from build123d import *

# Parameters (mm, degrees)
SKETCH1_R           = 17.5
BOSS_EXTRUDE1_DEPTH = 200
SKETCH3_OUTSIDE_W   = 78.206
SKETCH3_OUTSIDE_H   = 78.206
SKETCH3_OUTSIDE_R   = 12
CUT_EXTRUDE1_DEPTH  = 24
SKETCH4_W           = 220
SKETCH4_H           = 26
BOSS_EXTRUDE2_DEPTH = 23
CHAMFER1_SIZE       = 10


with BuildPart() as part:
    # Sketch1 → Boss-Extrude1 (new body)
    with BuildSketch(Plane.XY):
        Circle(SKETCH1_R)
    extrude(amount=BOSS_EXTRUDE1_DEPTH)

    # Sketch3 outside → Cut-Extrude1 (cut)
    with BuildSketch(Plane.XY.offset(200)):
        Rectangle(SKETCH3_OUTSIDE_W, SKETCH3_OUTSIDE_H)
        Circle(SKETCH3_OUTSIDE_R, mode=Mode.SUBTRACT)
    extrude(amount=-CUT_EXTRUDE1_DEPTH, mode=Mode.SUBTRACT)

    # Sketch4 → Boss-Extrude2 (add)
    with BuildSketch(Plane.XY.offset(200)):
        Rectangle(SKETCH4_W, SKETCH4_H)
    extrude(amount=BOSS_EXTRUDE2_DEPTH)

    # Chamfer1
    chamfer1_edges = [part.edges().sort_by_distance(p)[0] for p in [
        (-110, 0, 223),
        (110, 0, 223),
    ]]
    chamfer(chamfer1_edges, length=CHAMFER1_SIZE)


solid = part.part
The model under review builds one solid part; all positions refer to its coordinate system, in mm. A direction names the side the tool comes from. Give positions to 0.01 mm unless a question says otherwise; leave off trailing zeros. Loops run counter-clockwise (first coordinate to the right, second up) from the corner with the lowest first, then second, coordinate; pieces in that order, holes last. Notation, with made-up numbers: (67, 3.5) -> (125, 3.5) arc R12 cw to (125, 23.5) -> close; hole circle Ø7 at (75.5, -26.5). An arc over 180 degrees is marked (long way). Put each result on its own line as item: value. Start each with the question number.
1. We need section B-B on y = 5. State the section outline as (x, z) points.
2. Mouldability with a two-part tool opening along Z and no side actions: class faces 1 (the face through (-11.99, 0.53, 188.17)), 2 (the face through (0, 0, 0)), 3 (the face through (-13.887, -10.648, 86.768)) as released by +Z, released by -Z, zero draft, split by the parting line, or undercut.
3. For faces 4 (the face through (-105, 0, 218)), 5 (the face through (-12, -4, 176)), list the 3-axis set-ups (+Z, -Z, +X, -X, +Y, -Y) from which the entire face can be reached by the end or side of a thin tool; tool diameter is ignored.
4. We need section A-A on x = 0. State the section outline as (y, z) points.
5. We need section C-C on z = 125. State the section outline as (x, y) points.
6. Clearance check with flat-ended pins moving along their axes: P1, Ø1, axis at x = 78, y = -4, coming from the -Z side; P2, Ø11.5, axis at x = 14.5, z = 215.5, coming from the -Y side; P3, Ø1, axis at y = -13.5, z = 174, coming from the +X side. State where each tip first meets the part, or that it passes through.
7. We need section D-D on x = 34. State the section outline as (y, z) points.
8. Wall thickness on probe 1 along Z at (x, y) = (-62, -5); probe 2 along Y at (x, z) = (-7.5, 135.5); probe 3 along X at (y, z) = (4, 11.5): over which ranges is each line inside the solid? List them lowest first.
Determined:
1. outline: (-110, 200) -> (-10.91, 200) -> (-10.91, 176) -> (-16.77, 176) -> (-16.77, 0) -> (16.77, 0) -> (16.77, 176) -> (10.91, 176) -> (10.91, 200) -> (110, 200) -> (110, 213) -> (100, 223) -> (-100, 223) -> (-110, 213) -> close
2. face 1: undercut
2. face 2: released by -Z
2. face 3: zero draft
3. face 4: +Z, -X, +Y, -Y
3. face 5: none
4. outline: (-17.5, 0) -> (17.5, 0) -> (17.5, 176) -> (12, 176) -> (12, 200) -> (13, 200) -> (13, 223) -> (-13, 223) -> (-13, 200) -> (-12, 200) -> (-12, 176) -> (-17.5, 176) -> close
5. outline: circle Ø35 at (0, 0)
6. P1: z = 200
6. P2: y = -13
6. P3: x = 11.72
7. outline: (-13, 200) -> (13, 200) -> (13, 223) -> (-13, 223) -> close
8. probe 1: 200 to 223
8. probe 2: -15.81 to 15.81
8. probe 3: -17.04 to 17.04
